```python
from build123d import *

# Parameters (mm, degrees)
BOSS_EXTRUDE1_DEPTH = 20
SHELL1_T            = -2
CUT_EXTRUDE1_REACH  = 55.677
CUT_EXTRUDE2_REACH  = 55.677


with BuildPart() as part:
    # Sketch1 → Boss-Extrude1 (new body)
    with BuildSketch(Plane.XY):
        with BuildLine():
            Line((-32.851981106, 24.914801572), (-18.2983008, -8.072929322))
            ThreePointArc((-18.2983008, -8.072929322), (12.528602689, -15.589551458), (11.821088788, 16.132633383))
            Line((11.821088788, 16.132633383), (-17.262429648, 37.443404261))
            Line((-17.262429648, 37.443404261), (-32.851981106, 24.914801572))
        make_face()
    extrude(amount=BOSS_EXTRUDE1_DEPTH)

    # Shell1
    shell1_openings = [part.faces().sort_by_distance(p)[0] for p in [
        (-25.057205377, 31.179102917, 10),
    ]]
    offset(amount=SHELL1_T, openings=shell1_openings, kind=Kind.INTERSECTION)

    # Sketch2 → Cut-Extrude1 (cut, up to next)
    with BuildSketch(Plane(origin=(0, 0, 0), x_dir=(-1, 0, 0), z_dir=(0, 0, -1)), mode=Mode.PRIVATE) as cut_extrude1_sk1:
        Polygon((21.131336752, 21.505036784), (16.454471314, 25.263617591), (28.983074003, 40.853169049), (33.65993944, 37.094588242), align=None)
    cut_extrude1_tool1 = extrude(cut_extrude1_sk1.sketch, amount=-CUT_EXTRUDE1_REACH, mode=Mode.PRIVATE) & part.part
    add(cut_extrude1_tool1.solids().sort_by_distance((-25.057205, 31.179103, 0))[0], mode=Mode.SUBTRACT)

    # Sketch3 → Cut-Extrude2 (cut, up to next)
    with BuildSketch(Plane.XY.offset(20), mode=Mode.PRIVATE) as cut_extrude2_sk1:
        Polygon((-18.011864488, 24.008813734), (-512.566768876, 639.391815534), (-514.125724022, 638.138955265), (-19.570819634, 22.755953465), align=None)
    cut_extrude2_tool1 = extrude(cut_extrude2_sk1.sketch, amount=-CUT_EXTRUDE2_REACH, mode=Mode.PRIVATE) & part.part
    add(cut_extrude2_tool1.solids().sort_by_distance((-266.068794, 331.073884, 20))[0], mode=Mode.SUBTRACT)


solid = part.part
```
Model file for the job. Use its own axes, mm. A direction names the side the tool comes from. Coordinates: 2 decimals unless noted, no trailing zeros. Loops run counter-clockwise (first coordinate to the right, second up) from the corner with the lowest first, then second, coordinate; pieces in that order, holes last. Notation, with made-up numbers: (75, 68) - (80, 68) arc R16 ccw to (80, 99) - close; hole circle Ø1 at (53.5, -5). An arc over 180 degrees is marked (long way). Write item = value, one per line. Start each with the question number.
Item 1: 3-axis set-ups, long thin cutter, end or side, ignore diameter. For faces 1 (the face through (-7, 9, 0)), 2 (the face through (-22.75, 26.71, 19.01)), 3 (the face through (-2.52, 26.64, 9.86)), 4 (the face through (-3.91, 25.18, 9.89)), 5 (the face through (-18.826, 23.358, 0.986)): which of +Z, -Z, +X, -X, +Y, -Y reach the whole face in a straight line?
Item 2: Wall check: probe 1 along Z at (x, y) = (-27.5, 29); probe 2 along Y at (x, z) = (16, 4.5); probe 3 along Y at (x, z) = (-9, 12.5). Give the ranges that are in metal, low to high. Write a range as [from, to].
Item 3: Saw through at C-C, the plane z = 12. List the corners of the cut face in (x, y).
Item 4: Drop flat-ended pins along their axis: pin 1 Ø5 at (y, z) = (-11.5, 11) entering from -X; pin 2 Ø4 at (y, z) = (11, 4) entering from -X; pin 3 Ø8 at (y, z) = (-4.5, 15.5) entering from -X. Give the stop position or say it passes through.
Item 5: Saw through at A-A, the plane x = -14. List the corners of the cut face in (y, z), then the cut area to 3 significant figures.
Item 6: Saw through at D-D, the plane y = 34.5. List the corners of the cut face in (x, z), then the cut area to 3 significant figures.
Item 7: Pull direction Y, two halves, no side cores. Call faces 6 (the face through (-25.7, 8.7, 9.9)), 7 (the face through (-31.634, 25.894, 9.86)), 8 (the face through (10.912, -14.315, 9.888)), 9 (the face through (12, -16, 10)): +Y half, -Y half, draft (parallel to the pull), parting line (faces both ways), or undercut.
Item 8: Saw through at B-B, the plane y = 2. List the corners of the cut face in (x, z), then the cut area to 3 significant figures.
Answers:
q1.face_1 = -Z, +X, -X, +Y, -Y
q1.face_2 = +Z, -Z
q1.face_3 = +Z, -Z, +X, +Y
q1.face_4 = none
q1.face_5 = -Z
q2.probe_1 = [0, 2], [18, 20]
q2.probe_2 = [-12, -8.25], [8.25, 12]
q2.probe_3 = [-17.86, -15.59], [28.91, 31.39]
q3.outline = (-32.85, 24.91) - (-18.3, -8.07) arc R20 ccw (long way) to (11.82, 16.13) - (-17.26, 37.44) - (-18.88, 36.15) - (10.64, 14.52) arc R18 cw (long way) to (-16.47, -7.27) - (-31.24, 26.21) - close
q4.pin_1 = -17.86
q4.pin_2 = -27.6
q4.pin_3 = -21.64
q5.outline = (-14.28, 0) - (35.05, 0) - (35.05, 20) - (-14.28, 20) - close; hole (-11.31, 2) - (32.57, 2) - (32.57, 18) - (-11.31, 18) - close
q5.area = 285 mm2
q6.outline = (-20.92, 0) - (-13.25, 0) - (-13.25, 20) - (-20.92, 20) - (-20.92, 18) - (-16.63, 18) - (-16.63, 2) - (-20.92, 2) - close
q6.area = 84.9 mm2
q7.face_6 = -Y half
q7.face_7 = +Y half
q7.face_8 = undercut
q7.face_9 = parting line
q8.outline = (-22.74, 0) - (19.9, 0) - (19.9, 20) - (-22.74, 20) - close; hole (-20.56, 2) - (17.89, 2) - (17.89, 18) - (-20.56, 18) - close
q8.area = 238 mm2
